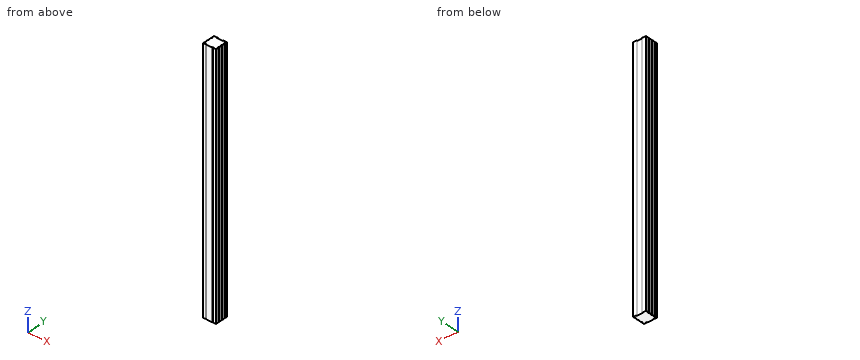
```python
from build123d import *

# Parameters (mm, degrees)
SKETCH_1_W               = 75
SKETCH_1_H               = 75
EXTRUDE_1_DEPTH          = 732.5
CUT_EXTRUDE_1_DEPTH      = 732.5
CUT_EXTRUDE_2_DEPTH      = 1465
CUT_EXTRUDE_3_DEPTH      = 1466.959583345
CUT_EXTRUDE_3_DEPTH_BACK = 1466.959583345


with BuildPart() as part:
    # 草图1 → 凸台-拉伸1 (new, symmetric)
    with BuildSketch(Plane.XY):
        Rectangle(SKETCH_1_W, SKETCH_1_H)
    extrude(amount=EXTRUDE_1_DEPTH, both=True)

    # 草图2 → 切除-拉伸1 (cut, symmetric)
    with BuildSketch(Plane.XY):
        Polygon((-17.9, -36.8), (-16.55, -36.8), (-16.55, -34.5), (-25.45, -34.5), (-25.45, -36.8), (-24.1, -36.8), (-24.1, -37.5), (-17.9, -37.5), align=None)
        Polygon((16.55, -34.5), (16.55, -36.8), (17.9, -36.8), (17.9, -37.5), (24.1, -37.5), (24.1, -36.8), (25.45, -36.8), (25.45, -34.5), align=None)
    extrude(amount=CUT_EXTRUDE_1_DEPTH, both=True, mode=Mode.SUBTRACT)

    # 草图3 → 切除-拉伸2 (cut)
    with BuildSketch(Plane.XY.offset(732.5)):
        Polygon((37.5, 2.6), (36.8, 2.6), (36.8, 4.45), (34.5, 4.45), (34.5, -4.45), (36.8, -4.45), (36.8, -2.6), (37.5, -2.6), align=None)
        Polygon((37.5, -17.9), (36.8, -17.9), (36.8, -16.55), (34.5, -16.55), (34.5, -25.45), (36.8, -25.45), (36.8, -24.1), (37.5, -24.1), align=None)
        Polygon((36.8, 24.1), (36.8, 25.45), (34.5, 25.45), (34.5, 16.55), (36.8, 16.55), (36.8, 17.9), (37.5, 17.9), (37.5, 24.1), align=None)
    cut_extrude_2 = extrude(amount=-CUT_EXTRUDE_2_DEPTH, mode=Mode.SUBTRACT)

    # 镜向1: 切除-拉伸2 across plane
    add(cut_extrude_2.mirror(Plane(origin=(0, 0, 0), x_dir=(0, 0, 1), z_dir=(1, 0, 0))), mode=Mode.SUBTRACT)

    # 草图4 → 切除-拉伸3 (cut, two sides: drawn at the far end of the back side and taken through both)
    with BuildSketch(Plane.XY.offset(732.5).offset(-CUT_EXTRUDE_3_DEPTH_BACK)):
        Polygon((164.287302387, 109.214920955), (-15, 37.5), (-25, 33.5), (25, 33.5), (15, 37.5), (-164.287302387, 109.214920955), (-164.287302387, -276.981747517), (164.287302387, -276.981747517), align=None)
    extrude(amount=CUT_EXTRUDE_3_DEPTH + CUT_EXTRUDE_3_DEPTH_BACK, mode=Mode.SUBTRACT)


solid = part.part
```
Check sheet for the modelled part. Datum: model origin and axes. Units: mm. Coordinates: 2 decimals unless noted, no trailing zeros. Loops run counter-clockwise (first coordinate to the right, second up) from the corner with the lowest first, then second, coordinate; pieces in that order, holes last.
1) Sectioned sample at A-A (x = -3). Record the boundary of the cut face in (y, z), and give its area (3 significant figures).
2) Gauge pin test, flat ends, axial feed: pin 1 (1 mm diameter, centred on y = -18.5, z = -407.5, fed in from -X); pin 2 (7 mm diameter, centred on y = 0, z = -70, fed in from +X); pin 3 (2 mm diameter, centred on y = -20.5, z = -379.5, fed in from +X). Record the tip position at first contact, or that the pin passes through.
3) Material ranges on probe 1 along X at (y, z) = (-24.5, 21); probe 2 along Y at (x, z) = (-6, 73.5); probe 3 along Y at (x, z) = (18.5, 539.5), recorded low to high.
Check sheet entries:
1. outline: (-37.5, -732.5) - (33.5, -732.5) - (33.5, 732.5) - (-37.5, 732.5) - close
1. area: 104,000 mm2
2. pin 1: stops at x = -34.5
2. pin 2: stops at x = 37.5
2. pin 3: stops at x = 34.5
3. probe 1: x = -37.5 to -36.8, -34.5 to 34.5, 36.8 to 37.5
3. probe 2: y = -37.5 to 33.5
3. probe 3: y = -34.5 to 33.5, 36.1 to 37.5
